Geometry: see drawing. Coordinates: mm, zero at the bounding-box minimum. A direction names the side the tool comes from. Give positions to 0.01 mm unless a question says otherwise; leave off trailing zeros. Order: outer loops, then holes, each group sorted by start corner. A loop starts at its lowest first (then second) coordinate and runs counter-clockwise, first axis right, second up. Notation, with made-up numbers: M -9,-22.75 L 18,-22.75 A10 cw 18,-4.75 Z; hole C 7,-26.5 d4. An arc over 180 degrees is marked long. Answer as a JSON object with one key per item and string values. Group by question number.
1. Section query C-C (y = 130). Output: boundary loops of the cut face in (x, z), plus the area to 3 significant figures.
2. Pull-direction query (X, two-part tool) for the marked faces 3, 4 and 5; classes: +X half, -X half, draft (parallel to the pull), parting line (faces both ways), or undercut.
3. Set-up query: the marked faces 1 and 2. Return all of +Z, -Z, +X, -X, +Y, -Y with unobstructed straight access to the full face (end or side cutting, diameter ignored); none if empty.
4. Section query A-A (y = 63.5). Output: boundary loops of the cut face in (x, z), plus the area to 3 significant figures.
5. Section query B-B (z = 22.5). Output: boundary loops of the cut face in (x, y).
6. Pin query (flat end, axial travel): P1, Ø13, axis at y = 130, z = 22.5, coming from the +X side; P2, Ø6.5, axis at x = 13, z = 33.5, coming from the +Y side. Return the tip coordinate at first contact, or that it passes through.
7. Section query D-D (z = 39.5). Output: boundary loops of the cut face in (x, y), plus the area to 3 significant figures.
8. Material intervals for L1, parallel to X at y = 9, z = 17; L2, parallel to Y at x = 1, z = 22; L3, parallel to Y at x = 30.6, z = 22.5, sorted ascending. Write a range as [from, to].
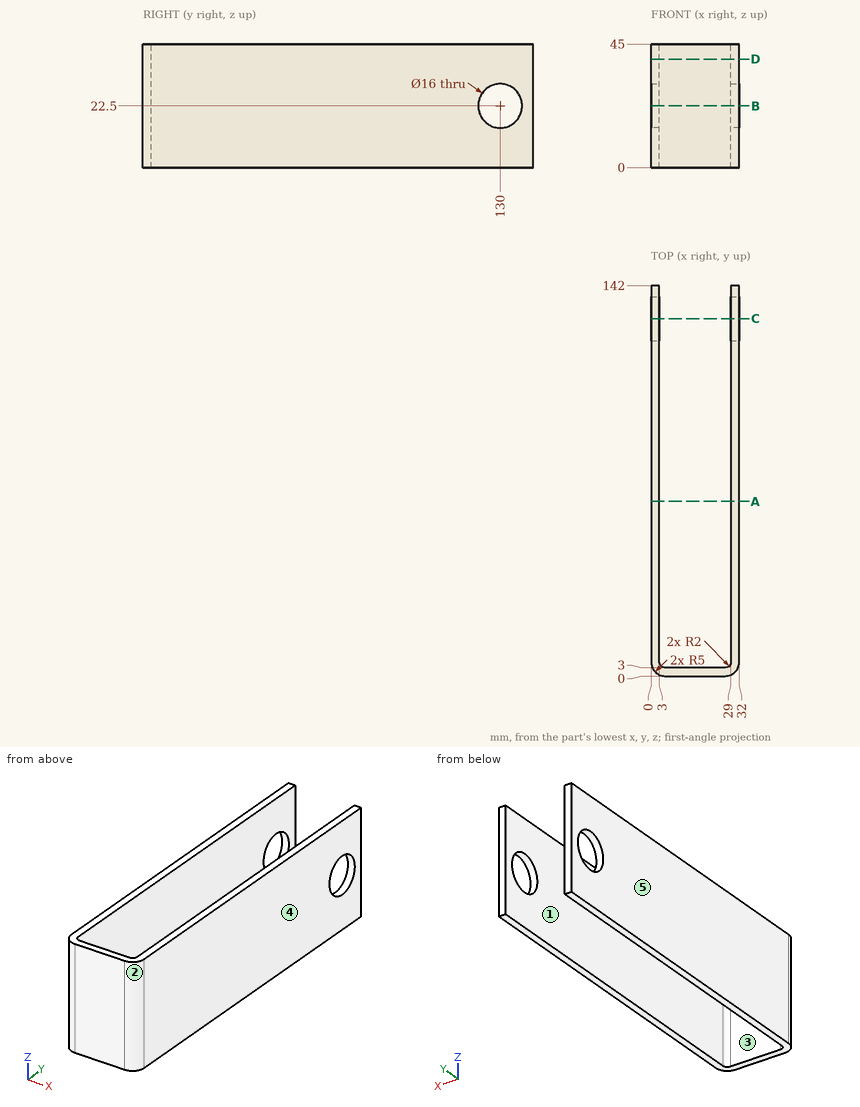
Answer sheet:
{
 "1": {"outline": "M 0,0 L 3,0 L 3,14.5 L 0,14.5 Z; M 0,30.5 L 3,30.5 L 3,45 L 0,45 Z; M 29,0 L 32,0 L 32,14.5 L 29,14.5 Z; M 29,30.5 L 32,30.5 L 32,45 L 29,45 Z", "area": "174 mm^2"},
 "2": {"face 3": "undercut", "face 4": "+X half", "face 5": "-X half"},
 "3": {"face 1": "+Z, -Z, +Y", "face 2": "+Z, -Z, +X, -Y"},
 "4": {"outline": "M 0,0 L 3,0 L 3,45 L 0,45 Z; M 29,0 L 32,0 L 32,45 L 29,45 Z", "area": "270 mm^2"},
 "5": {"outline": "M 0,5 A5 ccw 5,0 L 27,0 A5 ccw 32,5 L 32,122 L 29,122 L 29,5 A2 cw 27,3 L 5,3 A2 cw 3,5 L 3,122 L 0,122 Z; M 0,138 L 3,138 L 3,142 L 0,142 Z; M 29,138 L 32,138 L 32,142 L 29,142 Z"},
 "6": {"P1": "through", "P2": "y = 3"},
 "7": {"outline": "M 0,5 A5 ccw 5,0 L 27,0 A5 ccw 32,5 L 32,142 L 29,142 L 29,5 A2 cw 27,3 L 5,3 A2 cw 3,5 L 3,142 L 0,142 Z", "area": "921 mm^2"},
 "8": {"L1": "[0, 3], [29, 32]", "L2": "[2, 122.02], [137.98, 142]", "L3": "[1.53, 122], [138, 142]"}
}
